Can you work these out from the drawing? Everything is in mm from the part's minimum corner. A direction names the side the tool comes from. Give positions to 0.01 mm unless a question says otherwise; leave off trailing zeros. Write each loop counter-clockwise with the first axis right and the second up, starting at its lowest first coordinate (ties: lowest second). Pieces come first, ordered by that corner, then holes. Notation, with made-up numbers: (47.25, -36) - (65.25, -36) arc R7 ccw to (65.25, -31) - close; hole circle Ø8 at (84.25, 1). An arc over 180 degrees is marked (long way). Answer in a Markdown table with one row per item.
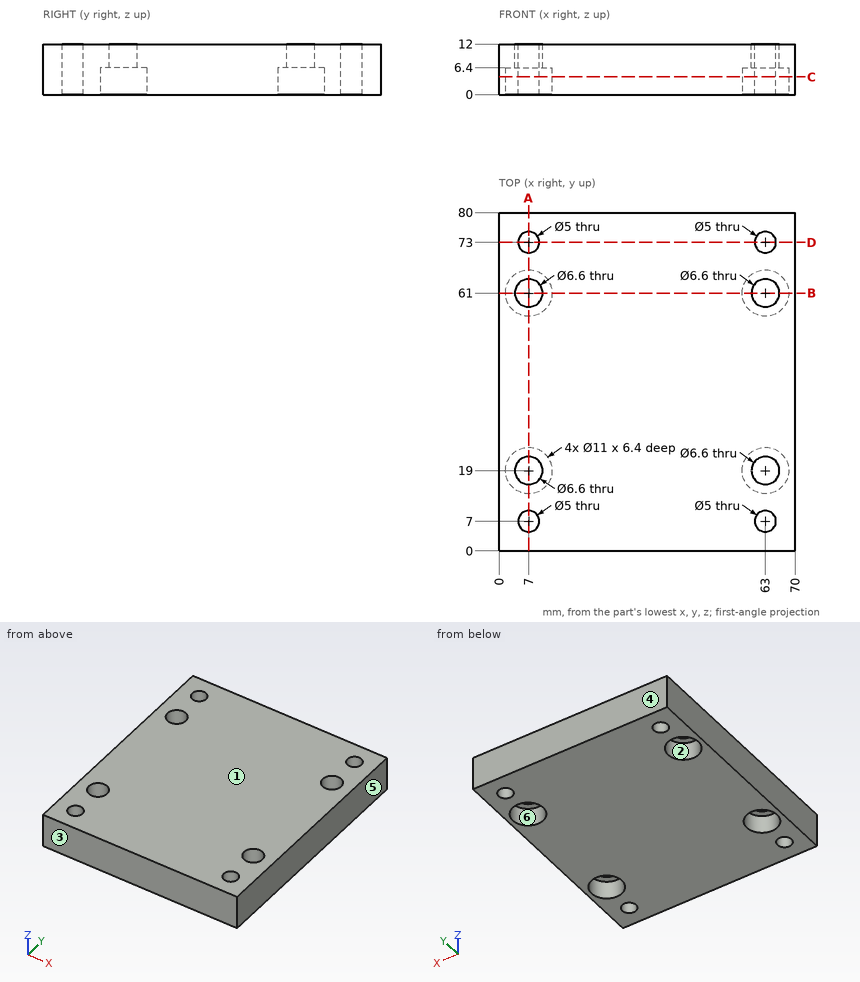
1) Will this pin go through, and if not, where does the flat tip stop? P1, Ø8.5, axis at x = 63, y = 61, coming from the -Z side.
Check values:
| item | result |
|---|---|
| P1 | stops at z = 6.4 |
2) Imagine slicing it at A-A (x = 7). List the corners of the cut face in (y, z) for me, then the cut area to 3 significant figures.
Check values:
| item | result |
|---|---|
| outline | (0, 0) - (4.5, 0) - (4.5, 12) - (0, 12) - close; (9.5, 0) - (13.5, 0) - (13.5, 6.4) - (15.7, 6.4) - (15.7, 12) - (9.5, 12) - close; (22.3, 6.4) - (24.5, 6.4) - (24.5, 0) - (55.5, 0) - (55.5, 6.4) - (57.7, 6.4) - (57.7, 12) - (22.3, 12) - close; (64.3, 6.4) - (66.5, 6.4) - (66.5, 0) - (70.5, 0) - (70.5, 12) - (64.3, 12) - close; (75.5, 0) - (80, 0) - (80, 12) - (75.5, 12) - close |
| area | 625 mm2 |
3) If I drill on line 1 (Y direction, x = 63, z = 10.8); line 2 (Y direction, x = 63, z = 2.75); line 3 (X direction, y = 64, z = 3.75), over which ranges is the centre line in solid material (lowest first)?
Check values:
| item | result |
|---|---|
| line 1 | y = 0 to 4.5, 9.5 to 15.7, 22.3 to 57.7, 64.3 to 70.5, 75.5 to 80 |
| line 2 | y = 0 to 4.5, 9.5 to 13.5, 24.5 to 55.5, 66.5 to 70.5, 75.5 to 80 |
| line 3 | x = 0 to 2.39, 11.61 to 58.39, 67.61 to 70 |
4) Imagine slicing it at C-C (z = 4.25). State how many separate pieces and enclosed holes the cut face has, then the cut area to 3 significant figures.
Check values:
| item | result |
|---|---|
| separate pieces | 1 |
| enclosed holes | 8 |
| area | 5,140 mm2 |
5) Imagine slicing it at B-B (y = 61). List the corners of the cut face in (x, z) for me.
Check values:
| item | result |
|---|---|
| outline | (0, 0) - (1.5, 0) - (1.5, 6.4) - (3.7, 6.4) - (3.7, 12) - (0, 12) - close; (10.3, 6.4) - (12.5, 6.4) - (12.5, 0) - (57.5, 0) - (57.5, 6.4) - (59.7, 6.4) - (59.7, 12) - (10.3, 12) - close; (66.3, 6.4) - (68.5, 6.4) - (68.5, 0) - (70, 0) - (70, 12) - (66.3, 12) - close |
6) We'd pull the mould along Y, two halves only. Please class the marked faces 1, 2, 3 and 4: +Y half, -Y half, draft (parallel to the pull), parting line (faces both ways), or undercut.
Check values:
| item | result |
|---|---|
| face 1 | draft |
| face 2 | undercut |
| face 3 | -Y half |
| face 4 | +Y half |
7) On a 3-axis mill with a long thin cutter (end or side, diameter ignored), from which of +Z, -Z, +X, -X, +Y, -Y can I reach the whole of each face in a straight line? I mean the marked faces 5 and 6. Say none if no direction works.
Check values:
| item | result |
|---|---|
| face 5 | +Z, -Z, +X, +Y, -Y |
| face 6 | -Z |
8) Imagine slicing it at D-D (y = 73). List the corners of the cut face in (x, z) for me, then the cut area to 3 significant figures.
Check values:
| item | result |
|---|---|
| outline | (0, 0) - (4.5, 0) - (4.5, 12) - (0, 12) - close; (9.5, 0) - (60.5, 0) - (60.5, 12) - (9.5, 12) - close; (65.5, 0) - (70, 0) - (70, 12) - (65.5, 12) - close |
| area | 720 mm2 |
